The listing builds one solid part. Answer for the finished solid, in the listing's coordinates (mm). A direction names the side the tool comes from. Coordinates: 2 decimals unless noted, no trailing zeros. Order: outer loops, then holes, each group sorted by start corner. A loop starts at its lowest first (then second) coordinate and runs counter-clockwise, first axis right, second up. Notation, with made-up numbers: (55, -21.75) -> (110, -21.75) arc R16 ccw to (110, 8.25) -> close; hole circle Ø5 at (54.25, 47). An arc over 180 degrees is marked (long way). Return JSON: item names as keys, results as strings.
from build123d import *


with BuildPart() as part:
    # 草图1 → 旋转1 (revolve)
    with BuildSketch(Plane.XY, mode=Mode.PRIVATE) as revolve_1_sk:
        Polygon((0, 0), (0, 27.5), (40, 27.5), (40, 26.5), (42, 26.5), (42, 30), (532, 30), (532, 26.5), (572, 26.5), (572, 0), align=None)
    revolve(revolve_1_sk.sketch.rotate(Axis((0, 0, 0), (1, 0, 0)), 90), axis=Axis((0, 0, 0), (1, 0, 0)))


solid = part.part
1. The part is cut by section A-A on y = -19.5. Give the vertices of the cut face in (x, z), and give its area (3 significant figures).
Answer block:
{"outline": "(0, -19.39) -> (40, -19.39) -> (40, -17.94) -> (42, -17.94) -> (42, -22.8) -> (532, -22.8) -> (532, -17.94) -> (572, -17.94) -> (572, 17.94) -> (532, 17.94) -> (532, 22.8) -> (42, 22.8) -> (42, 17.94) -> (40, 17.94) -> (40, 19.39) -> (0, 19.39) -> close", "area": "25,400 mm2"}
2. For faces 1 (the face through (572, 0, 0)), 2 (the face through (20.28, 24.397, 12.69)), 3 (the face through (42, 27, 0)), determine the directions among +Z, -Z, +X, -X, +Y, -Y from which every point of the face is accessible in a straight line to the end or side of a thin tool.
Answer block:
{"face 1": "+Z, -Z, +X, +Y, -Y", "face 2": "-X", "face 3": "none"}
3. The part is cut by section C-C on x = 286. Give the vertices of the cut face in (y, z), and give its area (3 significant figures).
Answer block:
{"outline": "circle Ø60 at (0, 0)", "area": "2,830 mm2"}
4. Consider line 1 (Y direction, x = 317, z = -2.5); line 2 (Z direction, x = 300.5, y = -2); line 3 (Y direction, x = 431.5, z = 1.5). Determine where each line is inside the solid, lowest interval first. Write a range as from..to.
Answer block:
{"line 1": "y = -29.9..29.9", "line 2": "z = -29.93..29.93", "line 3": "y = -29.96..29.96"}
5. Determine the mould class of faces 4 (the face through (41.014, -26.274, -3.45)), 5 (the face through (552.28, -26.274, -3.45)), 6 (the face through (40, -23, -14)), 7 (the face through (532, 27, 0)) for opening direction X: pulls with the +X half, pulls with the -X half, needs draft (parallel to the pull), parting line crosses it, or undercut.
Answer block:
{"face 4": "undercut", "face 5": "needs draft", "face 6": "undercut", "face 7": "pulls with the +X half"}
6. The part is cut by section B-B on z = -5. Give the vertices of the cut face in (x, y).
Answer block:
{"outline": "(0, -27.04) -> (40, -27.04) -> (40, -26.02) -> (42, -26.02) -> (42, -29.58) -> (532, -29.58) -> (532, -26.02) -> (572, -26.02) -> (572, 26.02) -> (532, 26.02) -> (532, 29.58) -> (42, 29.58) -> (42, 26.02) -> (40, 26.02) -> (40, 27.04) -> (0, 27.04) -> close"}
7. Each of these flat-tipped pins is pushed along its axis until it touches: pin 1 Ø1 at (x, z) = (136.5, -14.5) entering from +Y; pin 2 Ø10 at (x, z) = (471.5, 10) entering from -Y; pin 3 Ø1.5 at (y, z) = (19.5, -22) entering from +X; pin 4 Ø18 at (y, z) = (-12, -5.5) entering from -X. Where does it stop, or does it pass through?
Answer block:
{"pin 1": "stops at y = 26.53", "pin 2": "stops at y = -29.58", "pin 3": "stops at x = 532", "pin 4": "stops at x = 0"}
